Here's how the part is built. I have some questions about the finished solid (model axes, mm). Face numbers are marked on the shaded views. A direction names the side the tool comes from. Coordinates: 2 decimals unless noted, no trailing zeros. Write each loop counter-clockwise with the first axis right and the second up, starting at its lowest first coordinate (ties: lowest second). Pieces come first, ordered by that corner, then holes.
Item 1: We'd pull the mould along X, two halves only. Please class the marked faces 6, 7 and 8: +X half, -X half, draft (parallel to the pull), parting line (faces both ways), or undercut.
Item 2: If we section it at B-B (y = -4): Please give me the cut outline in (x, z), then the cut area to 3 significant figures.
Item 3: If we section it at C-C (z = 0): Please give me the cut outline in (x, y), then the cut area to 3 significant figures.
Item 4: For the marked faces 1, 2, 3, 4 and 5, which set-ups out of +Z, -Z, +X, -X, +Y, -Y let a thin tool reach every point of the face, with its end or its side?
Item 5: If I drill on line 1 (Z direction, x = -1.5, y = -8.75); line 2 (X direction, y = -3, z = -2.25); line 3 (Z direction, x = 0, y = -6), over which ranges is the centre line in solid material (lowest first)?
Item 6: If we section it at A-A (z = 2.75): Please give me the cut outline in (x, y), then the cut area to 3 significant figures.
Item 7: If we section it at D-D (x = -1.75): Please give me the cut outline in (y, z).
Item 8: I'm going to push flat-ended pins straight in: pin 1 Ø1 at (x, z) = (1.5, 2.5) entering from +Y; pin 2 Ø1.4 at (x, y) = (-0.5, -5) entering from +Z; pin 3 Ø3 at (x, y) = (2.5, -3) entering from +Z. Where does each tip first touch, or does it pass through?
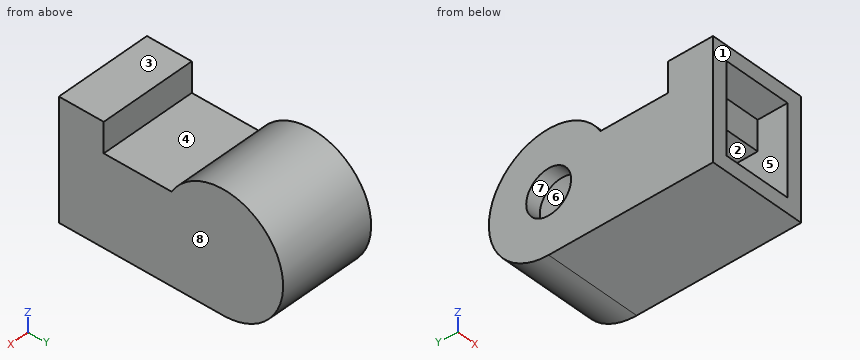
from build123d import *

# Parameters (mm, degrees)
LEG_BODY_DEPTH        = 3.25
LEG_SHELL_1MM_T       = -1
HIP_PIN_HOLE_3_REACH  = 15.388
HIP_PIN_HOLE_SKETCH_R = 1.5


with BuildPart() as part:
    # Leg Profile Sketch → Leg Body (new, symmetric)
    with BuildSketch(Plane(origin=(0, 0, 0), x_dir=(0, 0, -1), z_dir=(1, 0, 0))):
        with BuildLine():
            Line((4, 0), (4, -11))
            Line((4, -11), (-4, -11))
            Line((-4, -11), (-4, -8))
            Line((-4, -8), (-2, -8))
            Line((-2, -8), (-2, -3.464101615))
            ThreePointArc((-2, -3.464101615), (-2, 3.464101615), (4, 0))
        make_face()
    extrude(amount=LEG_BODY_DEPTH, both=True)

    # Leg Shell 1mm
    leg_shell_1mm_openings = [part.faces().sort_by_distance(p)[0] for p in [
        (0, -11, 0),
    ]]
    offset(amount=LEG_SHELL_1MM_T, openings=leg_shell_1mm_openings, kind=Kind.INTERSECTION)

    # Hip Pin Hole Sketch → Hip Pin Hole Ø3 (cut, up to next)
    with BuildSketch(Plane.ZY.offset(3.25), mode=Mode.PRIVATE) as hip_pin_hole_3_sk1:
        Circle(HIP_PIN_HOLE_SKETCH_R)
    hip_pin_hole_3_tool1 = extrude(hip_pin_hole_3_sk1.sketch, amount=-HIP_PIN_HOLE_3_REACH, mode=Mode.PRIVATE) & part.part
    add(hip_pin_hole_3_tool1.solids().sort_by_distance((-3.25, 0, 0))[0], mode=Mode.SUBTRACT)


solid = part.part
Answer list:
1. face 6: undercut
1. face 7: draft
1. face 8: +X half
2. outline: (-3.25, -4) - (3.25, -4) - (3.25, 2) - (-3.25, 2) - close; hole (-2.25, -3) - (2.25, -3) - (2.25, 1) - (-2.25, 1) - close
2. area: 21.0 mm2
3. outline: (-3.25, -11) - (-2.25, -11) - (-2.25, -1.5) - (-3.25, -1.5) - close; (-3.25, 1.5) - (-2.25, 1.5) - (-2.25, 3) - (2.25, 3) - (2.25, -11) - (3.25, -11) - (3.25, 4) - (-3.25, 4) - close
3. area: 31.5 mm2
4. face 1: +Z, -Z, +X, -X, -Y
4. face 2: -Y
4. face 3: +Z, +X, -X, +Y, -Y
4. face 4: +Z, +X, -X
4. face 5: none
5. line 1: z = -4 to -3, 1 to 4
5. line 2: x = -3.25 to -2.25, 2.25 to 3.25
5. line 3: z = -4 to -3, 1 to 2
6. outline: (-3.25, -11) - (-2.25, -11) - (-2.25, -9) - (2.25, -9) - (2.25, -11) - (3.25, -11) - (3.25, -8) - (-3.25, -8) - close; (-3.25, -2.9) - (3.25, -2.9) - (3.25, 2.9) - (-3.25, 2.9) - close; hole (-2.25, -1.2) - (2.25, -1.2) - (2.25, 1.2) - (-2.25, 1.2) - close
6. area: 37.5 mm2
7. outline: (-11, -4) - (0, -4) arc R4 ccw (long way) to (-3.46, 2) - (-8, 2) - (-8, 4) - (-11, 4) - (-11, 3) - (-9, 3) - (-9, 1) - (-2.83, 1) arc R3 cw (long way) to (0, -3) - (-11, -3) - close
8. pin 1: stops at y = 3.46
8. pin 2: stops at z = 2
8. pin 3: stops at z = 3.71
